Here's the drawing with two shaded views (mm, measured from the low corner). I have some questions. A direction names the side the tool comes from. Round coordinates to 2 decimals unless told otherwise and drop trailing zeros. Order: outer loops, then holes, each group sorted by start corner. A loop starts at its lowest first (then second) coordinate and runs counter-clockwise, first axis right, second up. Notation, with made-up numbers: (-38.5, -27) -> (-8.5, -27) arc R14 ccw to (-8.5, -7) -> close; hole circle Ø1 at (70, -21). An arc over 180 degrees is marked (long way). Answer in a Markdown table with one row per item.
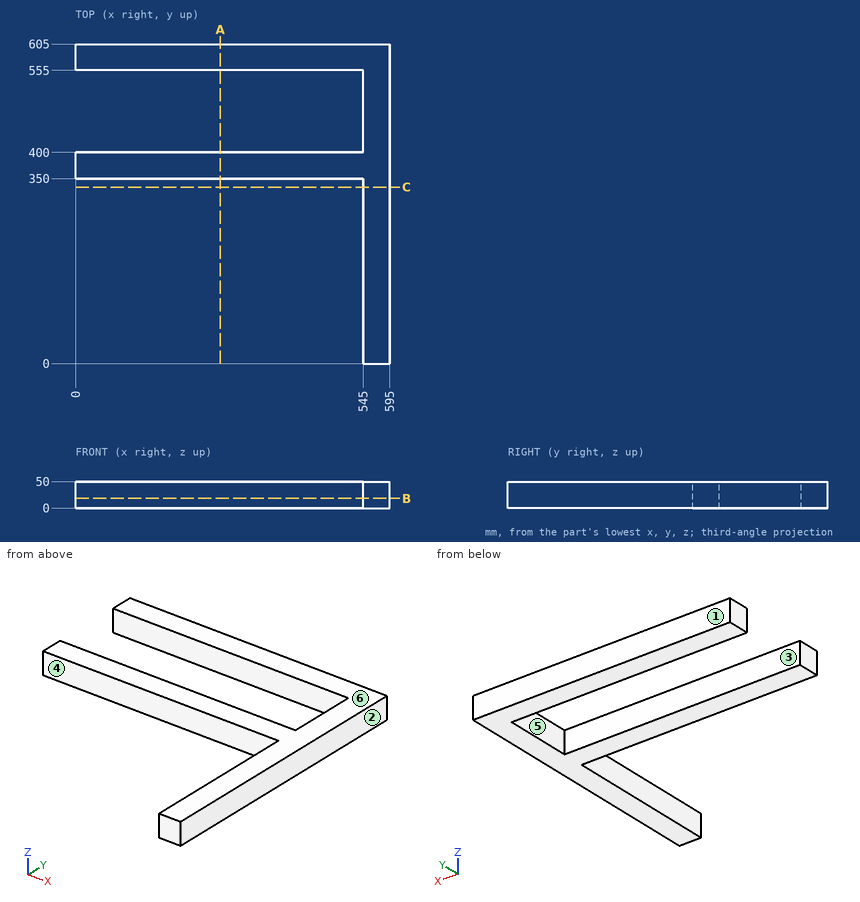
1. Please list where these lines run through material, in increasing order: line 1 along Y through (x, z) = (348, 21.5); line 2 along X through (y, z) = (529, 12).
Numbers:
| item | result |
|---|---|
| line 1 | y = 350 to 400, 555 to 605 |
| line 2 | x = 545 to 595 |
2. For pin 1 Ø3 at (y, z) = (86.5, 9.5) entering from -X; pin 2 Ø15 at (x, z) = (233.5, 30.5) entering from -Y, each with a flat end and sliding along its axis, tell me the tip position at first contact or that it passes through.
Numbers:
| item | result |
|---|---|
| pin 1 | stops at x = 545 |
| pin 2 | stops at y = 350 |
3. For the marked faces 4, 5 and 6, which set-ups out of +Z, -Z, +X, -X, +Y, -Y let a thin tool reach every point of the face, with its end or its side?
Numbers:
| item | result |
|---|---|
| face 4 | +Z, -Z, -X, -Y |
| face 5 | +Z, -Z, -X |
| face 6 | +Z, +X, -X, +Y, -Y |
4. Suppose I cut it at C-C on y = 334. Write out the boundary of the cut face in (x, z), then the cut area to 3 significant figures.
Numbers:
| item | result |
|---|---|
| outline | (545, 0) -> (595, 0) -> (595, 50) -> (545, 50) -> close |
| area | 2,500 mm2 |
5. We'd pull the mould along Y, two halves only. Please class the marked faces 1, 2 and 3: released by +Y, released by -Y, zero draft, split by the parting line, or undercut.
Numbers:
| item | result |
|---|---|
| face 1 | released by +Y |
| face 2 | zero draft |
| face 3 | undercut |
6. Suppose I cut it at B-B on z = 18.5. Write out the boundary of the cut face in (x, y), then the cut area to 4 significant figures.
Numbers:
| item | result |
|---|---|
| outline | (0, 350) -> (545, 350) -> (545, 0) -> (595, 0) -> (595, 605) -> (0, 605) -> (0, 555) -> (545, 555) -> (545, 400) -> (0, 400) -> close |
| area | 84,750 mm2 |
7. Suppose I cut it at A-A on x = 274. Write out the boundary of the cut face in (y, z).
Numbers:
| item | result |
|---|---|
| outline | (350, 0) -> (400, 0) -> (400, 50) -> (350, 50) -> close; (555, 0) -> (605, 0) -> (605, 50) -> (555, 50) -> close |
